Work out the finished part from the listing and answer in its coordinate system (mm). Face numbers are marked on the shaded views. Give positions to 0.01 mm unless a question says otherwise; leave off trailing zeros. Order: outer loops, then holes, each group sorted by start corner. A loop starts at its lowest first (then second) coordinate and runs counter-clockwise, first axis right, second up.
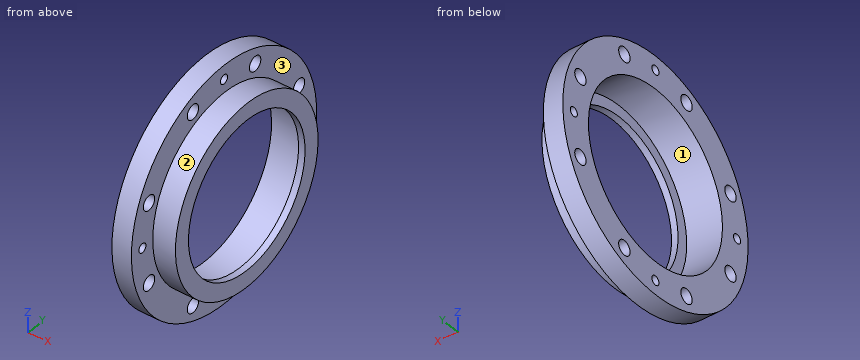
```python
from build123d import *

# Parameters (mm, degrees)
SKETCH2_R          = 11.22654111
CUT_EXTRUDE1_DEPTH = 30
CIRPATTERN1_COUNT  = 4


with BuildPart() as part:
    # Sketch1 → Revolve1 (revolve)
    with BuildSketch(Plane.XY, mode=Mode.PRIVATE) as revolve1_sk:
        Polygon((-79.177234861, 132), (-79.177234861, 182.5), (-49.177234861, 182.5), (-49.177234861, 140.5), (-14.177234861, 140.5), (-14.177234861, 114.860017889), (-24.177234861, 114.860017889), (-24.177234861, 132), align=None)
    revolve(revolve1_sk.sketch.rotate(Axis((-169.440966011, 0, 0), (1, 0, 0)), 90), axis=Axis((-169.440966011, 0, 0), (1, 0, 0)))

    # Sketch2 → Cut-Extrude1 (cut)
    with BuildSketch(Plane.ZY.offset(79.177234861)):
        with Locations((61.229349178, 147.820725202)):
            Circle(SKETCH2_R)
        with Locations((147.820725202, 61.229349178)):
            Circle(SKETCH2_R)
        with Locations((147.820725202, -61.229349178)):
            Circle(SKETCH2_R)
        with Locations((61.229349178, -147.820725202)):
            Circle(SKETCH2_R)
        with Locations((-61.229349178, -147.820725202)):
            Circle(SKETCH2_R)
        with Locations((-147.820725202, -61.229349178)):
            Circle(SKETCH2_R)
        with Locations((-147.820725202, 61.229349178)):
            Circle(SKETCH2_R)
        with Locations((-61.229349178, 147.820725202)):
            Circle(SKETCH2_R)
    extrude(amount=-CUT_EXTRUDE1_DEPTH, mode=Mode.SUBTRACT)

    # Sketch6 → M16 Tapped Hole1 (revolve, cut)
    with BuildSketch(Plane(origin=(-79.177234861, 160.836236417, 0), x_dir=(0, 0, 1), z_dir=(0, 1, 0))):
        Polygon((0, 0), (0, 46.206024333), (7, 42), (7, 0), align=None)
    m16_tapped_hole1 = revolve(axis=Axis((-85.527234861, 160.836236417, 0), (1, 0, 0)), mode=Mode.SUBTRACT)

    # CirPattern1: M16 Tapped Hole1 ×4 about axis
    cirpattern1_axis = Axis((0, 0, 0), (1, 0, 0))
    for i in range(1, CIRPATTERN1_COUNT):
        add(m16_tapped_hole1.rotate(cirpattern1_axis, i * 360 / CIRPATTERN1_COUNT), mode=Mode.SUBTRACT)


solid = part.part
```
1. The mould has two halves that part along Z. Classify the marked faces 1, 2 and 3: pulls with the +Z half, pulls with the -Z half, needs draft (parallel to the pull), parting line crosses it, or undercut.
Findings below:
face 1: undercut
face 2: parting line crosses it
face 3: needs draft
2. The part is cut by section C-C (x = -73.5). State how many separate pieces and enclosed holes the cut face has, then the cut area to 3 significant figures.
Findings below:
separate pieces: 1
enclosed holes: 13
area: 46,100 mm2
3. The part is cut by section A-A (z = 0). Write down the section's boundary in (x, y), then the cut area to 3 significant figures.
Findings below:
outline: (-79.18, -182.5) - (-49.18, -182.5) - (-49.18, -167.84) - (-79.18, -167.84) - close; (-79.18, -153.84) - (-49.18, -153.84) - (-49.18, -140.5) - (-14.18, -140.5) - (-14.18, -114.86) - (-24.18, -114.86) - (-24.18, -132) - (-79.18, -132) - close; (-79.18, 132) - (-24.18, 132) - (-24.18, 114.86) - (-14.18, 114.86) - (-14.18, 140.5) - (-49.18, 140.5) - (-49.18, 153.84) - (-79.18, 153.84) - close; (-79.18, 167.84) - (-49.18, 167.84) - (-49.18, 182.5) - (-79.18, 182.5) - close
area: 3,130 mm2
4. Straight lines are drawn through the part: probe 1 along Y at (x, z) = (-67, -0.5); probe 2 along Y at (x, z) = (-51, 0); probe 3 along Y at (x, z) = (-45, 0). For each, find the intervals that lie inside material, in ascending order.
Findings below:
probe 1: y = -182.5 to -167.82, -153.85 to -132, 132 to 153.85, 167.82 to 182.5
probe 2: y = -182.5 to -167.84, -153.84 to -132, 132 to 153.84, 167.84 to 182.5
probe 3: y = -140.5 to -132, 132 to 140.5
5. Given P1, Ø16, axis at y = 0, z = 160.84, coming from the +X side; P2, Ø8, axis at x = -34.5, z = -88, coming from the -Y side; P3, Ø3, axis at x = -42, y = -108, coming from the -Z side, each flat-ended and moving along its own axis, determine where each tip first touches the part or whether it passes through.
Findings below:
P1: stops at x = -49.18
P2: stops at y = -112.62
P3: stops at z = -91.64
6. The part is cut by section D-D (y = -88.5). Write down the section's boundary in (x, z), then the cut area to 3 significant figures.
Findings below:
outline: (-79.18, -159.61) - (-49.18, -159.61) - (-49.18, -109.12) - (-14.18, -109.12) - (-14.18, -73.22) - (-24.18, -73.22) - (-24.18, -97.94) - (-79.18, -97.94) - close; (-79.18, 97.94) - (-24.18, 97.94) - (-24.18, 73.22) - (-14.18, 73.22) - (-14.18, 109.12) - (-49.18, 109.12) - (-49.18, 159.61) - (-79.18, 159.61) - close
area: 4,980 mm2
